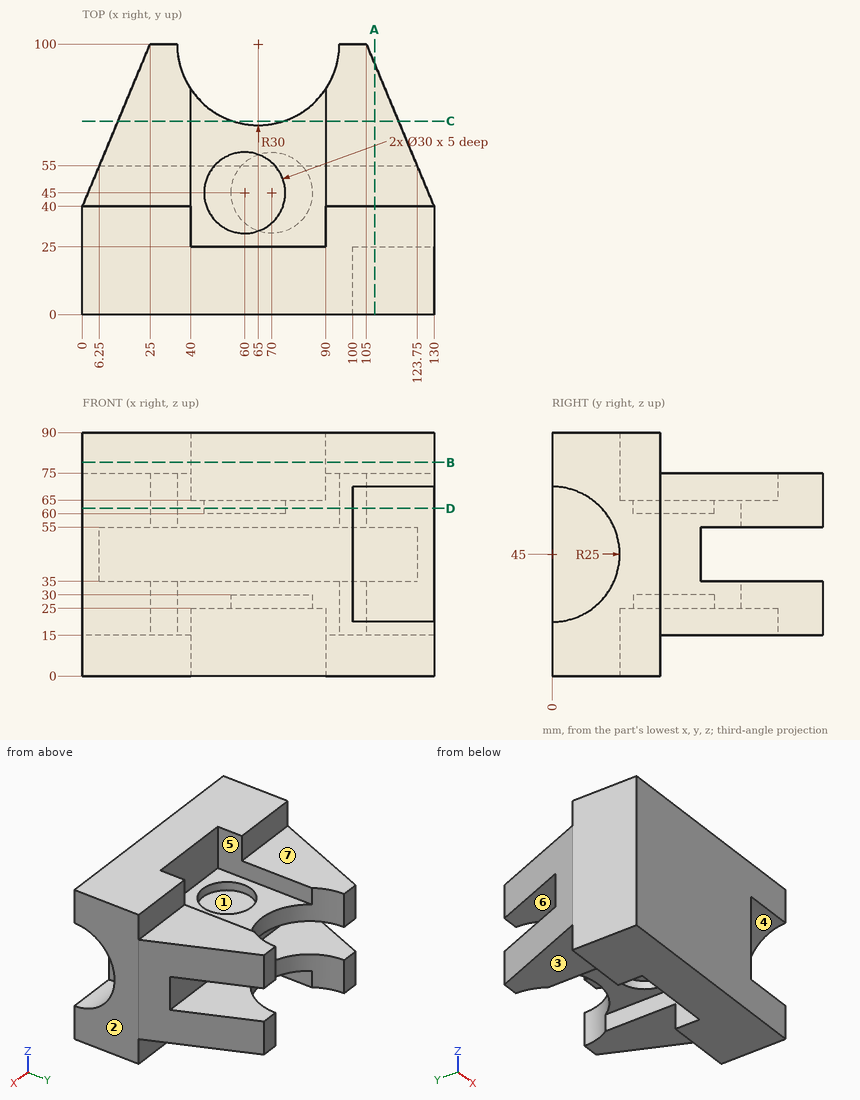
Here's the drawing with two shaded views (mm, measured from the low corner). I have some questions. A direction names the side the tool comes from. Coordinates: 2 decimals unless noted, no trailing zeros. Order: outer loops, then holes, each group sorted by start corner. A loop starts at its lowest first (then second) coordinate and runs counter-clockwise, first axis right, second up. Notation, with made-up numbers: M -25,29 L -19,29 A26 ccw -19,48 Z; hole C 2,70.25 d9. An arc over 180 degrees is marked long. Answer as CSV lines item,"result".
Item 1: Imagine slicing it at B-B on z = 79. Write out the boundary of the cut face in (x, y), plus the area to 3 significant figures.
Results found:
outline,"M 0,0 L 130,0 L 130,40 L 90,40 L 90,25 L 40,25 L 40,40 L 0,40 Z"
area,"4,450 mm2"
Item 2: On a 3-axis mill with a long thin cutter (end or side, diameter ignored), from which of +Z, -Z, +X, -X, +Y, -Y can I reach the whole of each face in a straight line? I mean the marked faces 5, 6 and 7. Say none if no direction works.
Results found:
face 5,"+Z, +Y"
face 6,"+X, -X, +Y"
face 7,"+Z, +X, -X, +Y"
Item 3: Imagine slicing it at D-D on z = 62. Write out the boundary of the cut face in (x, y), plus the area to 3 significant figures.
Results found:
outline,"M 0,0 L 100,0 L 100,18.33 L 130,18.33 L 130,40 L 105,100 L 95,100 A30 cw 35,100 L 25,100 L 0,40 Z; hole C 60,45 d30"
area,"8,830 mm2"
Item 4: For pin 1 (15 mm diameter, centred on x = 55.5, y = 58, fed in from +Z); pin 2 (1.5 mm diameter, centred on x = 14.5, z = 20.5, fed in from +Y); pin 3 (12 mm diameter, centred on y = 56, z = 67.5, fed in from +X), each with a flat end and sliding along its axis, tell me the tip position at first contact or that it passes through.
Results found:
pin 1,"z = 65"
pin 2,"y = 76.6"
pin 3,"x = 125.83"
Item 5: Imagine slicing it at C-C on y = 71.5. Write out the boundary of the cut face in (x, z) (1 decimal), plus the area to 3 significant figures.
Results found:
outline,"M 13.1,15 L 40,15 L 40,25 L 55.6,25 L 55.6,35 L 13.1,35 Z; M 13.1,55 L 55.6,55 L 55.6,65 L 40,65 L 40,75 L 13.1,75 Z; M 74.4,25 L 90,25 L 90,15 L 116.9,15 L 116.9,35 L 74.4,35 Z; M 74.4,55 L 116.9,55 L 116.9,75 L 90,75 L 90,65 L 74.4,65 Z"
area,"2,780 mm2"
Item 6: If I drill on line 1 (Z direction, x = 95.5, y = 56); line 2 (Y direction, x = 19.5, z = 40); line 3 (Y direction, x = 75, z = 18.5), over which ranges is the centre line in solid material (lowest first)?
Results found:
line 1,"15 to 35, 55 to 75"
line 2,"0 to 55"
line 3,"0 to 25"
Item 7: We'd pull the mould along Z, two halves only. Please class the marked faces 1, 2, 3 and 4: +Z half, -Z half, draft (parallel to the pull), parting line (faces both ways), or undercut.
Results found:
face 1,"+Z half"
face 2,"draft"
face 3,"-Z half"
face 4,"undercut"
Item 8: Imagine slicing it at A-A on x = 108. Write out the boundary of the cut face in (y, z), plus the area to 3 significant figures.
Results found:
outline,"M 0,0 L 40,0 L 40,15 L 92.8,15 L 92.8,35 L 55,35 L 55,55 L 92.8,55 L 92.8,75 L 40,75 L 40,90 L 0,90 L 0,70 A25 cw 0,20 Z"
area,"5,030 mm2"
